Here's how the part is built. I have some questions about the finished solid (model axes, mm). Coordinates: 2 decimals unless noted, no trailing zeros. Loops run counter-clockwise (first coordinate to the right, second up) from the corner with the lowest first, then second, coordinate; pieces in that order, holes last. Notation, with made-up numbers: (-6, 89.5) -> (1, 89.5) arc R18 cw to (1, 121.5) -> close; hole circle Ø3 at (-26.5, 75.25). An arc over 180 degrees is marked (long way). Answer as a JSON object with one key per item and string values. Group by question number.
1) I want a section at B-B (y = 0). Write out the boundary of the cut face in (x, z).
2) If we mould it in two halves opening along Y, with no side actions, what happens to faces 1 (the cylindrical face through (-1.08, -4.88, 9.86)), 2 (the flat face through (0, 7.5, 10)), 3 (the flat face through (-3, 5, 0))? For each: +Y half, -Y half, draft (parallel to the pull), parting line (faces both ways), or undercut.
3) I want a section at C-C (z = 17.5). Write out the boundary of the cut face in (x, y).
4) I want a section at A-A (x = 0). Write out the boundary of the cut face in (y, z), then the cut area to 3 significant figures.
5) I need wall thicknesses on probe 1 along Y at (x, z) = (0, 11.5); probe 2 along Y at (x, z) = (-2, 1); probe 3 along X at (y, z) = (-2.5, 16). Which ranges of each line are inside material? Lowest first, please. Write a range as [from, to].
```python
from build123d import *

# Parameters (mm, degrees)
SKETCH1_W           = 26
SKETCH1_H           = 15
SKETCH1_R           = 5
BOSS_EXTRUDE1_DEPTH = 20


with BuildPart() as part:
    # Sketch1 → Boss-Extrude1 (new body)
    with BuildSketch(Plane.XY):
        Rectangle(SKETCH1_W, SKETCH1_H)
        Circle(SKETCH1_R, mode=Mode.SUBTRACT)
    extrude(amount=BOSS_EXTRUDE1_DEPTH)


solid = part.part
```
Determined:
{
 "1": {"outline": "(-13, 0) -> (-5, 0) -> (-5, 20) -> (-13, 20) -> close; (5, 0) -> (13, 0) -> (13, 20) -> (5, 20) -> close"},
 "2": {"face 1": "undercut", "face 2": "+Y half", "face 3": "draft"},
 "3": {"outline": "(-13, -7.5) -> (13, -7.5) -> (13, 7.5) -> (-13, 7.5) -> close; hole circle Ø10 at (0, 0)"},
 "4": {"outline": "(-7.5, 0) -> (-5, 0) -> (-5, 20) -> (-7.5, 20) -> close; (5, 0) -> (7.5, 0) -> (7.5, 20) -> (5, 20) -> close", "area": "100 mm^2"},
 "5": {"probe 1": "[-7.5, -5], [5, 7.5]", "probe 2": "[-7.5, -4.58], [4.58, 7.5]", "probe 3": "[-13, -4.33], [4.33, 13]"}
}
